```python
from build123d import *

# Parameters (mm, degrees)
SKETCH_1_R      = 35
EXTRUDE_1_DEPTH = 10
SKETCH_2_R      = 15
EXTRUDE_2_DEPTH = 20
SKETCH_3_R      = 10
EXTRUDE_3_DEPTH = 100
SKETCH_4_R      = 9
EXTRUDE_4_DEPTH = 820
CHAMFER_1_SIZE  = 1
FILLET_1_R      = 10


with BuildPart() as part:
    # 草图1 → 凸台-拉伸1 (new body)
    with BuildSketch(Plane(origin=(0, 0, 0), x_dir=(0, 0, -1), z_dir=(1, 0, 0))):
        Circle(SKETCH_1_R)
    extrude(amount=EXTRUDE_1_DEPTH)

    # 草图2 → 凸台-拉伸2 (add)
    with BuildSketch(Plane(origin=(10, 0, 0), x_dir=(0, 0, -1), z_dir=(1, 0, 0))):
        Circle(SKETCH_2_R)
    extrude(amount=EXTRUDE_2_DEPTH)

    # 草图3 → 凸台-拉伸3 (add)
    with BuildSketch(Plane(origin=(30, 0, 0), x_dir=(0, 0, -1), z_dir=(1, 0, 0))):
        Circle(SKETCH_3_R)
    extrude(amount=EXTRUDE_3_DEPTH)

    # 草图4 → 凸台-拉伸4 (add)
    with BuildSketch(Plane(origin=(130, 0, 0), x_dir=(0, 0, -1), z_dir=(1, 0, 0))):
        with Locations(Location((0, 0, 0), (0, 0, 180))):
            Circle(SKETCH_4_R)
    extrude(amount=EXTRUDE_4_DEPTH)

    # 倒角1
    chamfer_1_edges = [part.edges().sort_by_distance(p)[0] for p in [
        (0, 0, 35),
        (10, 0, 35),
    ]]
    chamfer(chamfer_1_edges, length=CHAMFER_1_SIZE)

    # 圆角1
    fillet_1_edges = [part.edges().sort_by_distance(p)[0] for p in [
        (10, 0, 15),
    ]]
    fillet(fillet_1_edges, radius=FILLET_1_R)


solid = part.part
```
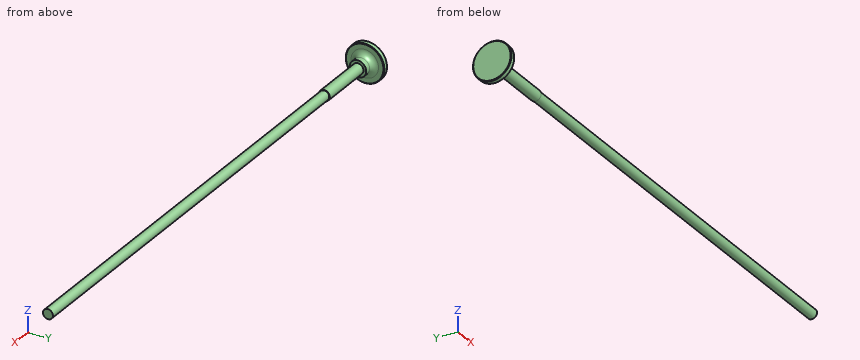
Geometry check sheet. Reference: the model listing, model coordinates, mm. Give positions to 0.01 mm unless a question says otherwise; leave off trailing zeros. Loops run counter-clockwise (first coordinate to the right, second up) from the corner with the lowest first, then second, coordinate; pieces in that order, holes last. Notation, with made-up numbers: (48, 33) - (99, 33) arc R23 ccw to (99, 64) - close; hole circle Ø8 at (2, 85). An arc over 180 degrees is marked (long way). Use CSV: the item, a comma, the result in double quotes. Start each with the question number.
Q1. Section check A-A, the plane y = 0. Record the cut outline in (x, z), and give its area (3 significant figures).
Q2. Scan lines: probe 1 along X at (y, z) = (0, -9.5); probe 2 along X at (y, z) = (-12, -5.5); probe 3 along Y at (x, z) = (667, -3.5). Record each from-to range of solid material in increasing order. Write a range as from..to.
Q3. Section check D-D, the plane x = 746. Record the cut outline in (y, z).
Q4. Go/stop test with flat-tipped pins: pin 1 Ø10 at (x, z) = (357, 4) entering from +Y; pin 2 Ø2 at (y, z) = (-20.5, 19) entering from +X; pin 3 Ø10 at (y, z) = (7, 22.5) entering from +X; pin 4 Ø8 at (x, y) = (409, -15) entering from +Z. Record where each tip stops, or that it passes through.
Q5. Section check C-C, the plane x = 61. Record the cut outline in (y, z).
Findings below:
1,outline,"(0, -34) - (1, -35) - (9, -35) - (10, -34) - (10, -25) arc R10 cw to (20, -15) - (30, -15) - (30, -10) - (130, -10) - (130, -9) - (950, -9) - (950, 9) - (130, 9) - (130, 10) - (30, 10) - (30, 15) - (20, 15) arc R10 cw to (10, 25) - (10, 34) - (9, 35) - (1, 35) - (0, 34) - close"
1,area,"18,100 mm^2"
2,probe 1,"x = 0..130"
2,probe 2,"x = 0..30"
2,probe 3,"y = -8.29..8.29"
3,outline,"circle Ø18 at (0, 0)"
4,pin 1,"stops at y = 9"
4,pin 2,"stops at x = 10"
4,pin 3,"stops at x = 12.35"
4,pin 4,"passes through"
5,outline,"circle Ø20 at (0, 0)"
